Check sheet for the modelled part. Datum: model origin and axes. Units: mm. A direction names the side the tool comes from. Coordinates: 2 decimals unless noted, no trailing zeros. Loops run counter-clockwise (first coordinate to the right, second up) from the corner with the lowest first, then second, coordinate; pieces in that order, holes last. Notation, with made-up numbers: (54, 26) -> (60, 26) arc R33 ccw to (60, 62) -> close; hole circle Ø7 at (27, 87). An arc over 180 degrees is marked (long way). Use CSV: the item, a comma, the result in double quotes.
```python
from build123d import *

# Parameters (mm, degrees)
BASE_EXTRUDE_DEPTH = 7.5
FILLET_2_R         = 0.6


with BuildPart() as part:
    # Sketch1 → Base-Extrude (new body)
    with BuildSketch(Plane(origin=(0, 0, 0), x_dir=(0, 0, -1), z_dir=(1, 0, 0))):
        Polygon((9, 5.196152423), (9, -5.196152423), (0, -10.392304845), (-9, -5.196152423), (-9, 5.196152423), (0, 10.392304845), align=None)
    extrude(amount=BASE_EXTRUDE_DEPTH)

    # Sketch2 → Boss-Revolve1 (revolve)
    with BuildSketch(Plane.XY, mode=Mode.PRIVATE) as boss_revolve1_sk:
        Polygon((0, 0), (77.5, 0), (77.5, 4.4845), (77.5, 6), (47.5, 6), (0, 6), align=None)
    revolve(boss_revolve1_sk.sketch.rotate(Axis((0, 0, 0), (1, 0, 0)), 90), axis=Axis((0, 0, 0), (1, 0, 0)))

    # Sketch3 → Cut-Revolve1 (revolve, cut)
    with BuildSketch(Plane.XY):
        Polygon((0, 9), (3.690598923, 15.392304845), (3.690598923, 20.392304845), (-10, 20.392304845), (-10, 9), align=None)
    revolve(axis=Axis((0, 0, 0), (1, 0, 0)), mode=Mode.SUBTRACT)

    # Sketch4 → Cut-Revolve3 (revolve, cut)
    with BuildSketch(Plane.XY, mode=Mode.PRIVATE) as cut_revolve3_sk:
        Polygon((7.5, 8.315), (6.9, 8.661410162), (6.9, 10.392304845), (7.5, 10.392304845), align=None)
    revolve(cut_revolve3_sk.sketch.rotate(Axis((0, 0, 0), (1, 0, 0)), 90), axis=Axis((0, 0, 0), (1, 0, 0)), mode=Mode.SUBTRACT)

    # Fillet 2
    fillet_2_edges = [part.edges().sort_by_distance(p)[0] for p in [
        (7.5, 0, -6),
    ]]
    fillet(fillet_2_edges, radius=FILLET_2_R)


solid = part.part
```
1) Access from +Z, -Z, +X, -X, +Y, -Y to the whole of each face (thin tool, end or side, straight path). Record for faces 1 (the flat face through (6.9, 8.4, 2.7)), 2 (the conical face through (0.195, 9.338, -0.023)).
Answer below:
face 1,"+X"
face 2,"-X, +Y"
2) Go/stop test with flat-tipped pins: pin 1 Ø1.5 at (x, z) = (67, -5.5) entering from -Y; pin 2 Ø1 at (x, z) = (44.5, -2) entering from +Y; pin 3 Ø4 at (x, z) = (64, 6.5) entering from +Y. Record where each tip stops, or that it passes through.
Answer below:
pin 1,"stops at y = -3.67"
pin 2,"stops at y = 5.81"
pin 3,"stops at y = 3.97"
3) Cross-section at A-A on x = 17.5. Record the boundary of the cut face in (y, z), and give its area (3 significant figures).
Answer below:
outline,"circle Ø12 at (0, 0)"
area,"113 mm²"
4) Thickness scan on line 1 along X through (y, z) = (7, 0); line 2 along Y through (x, z) = (31.5, 2.5); line 3 along Y through (x, z) = (22, 0). Record the ranges inside material, lowest first. Write a range as from..to.
Answer below:
line 1,"x = 0..7.5"
line 2,"y = -5.45..5.45"
line 3,"y = -6..6"
